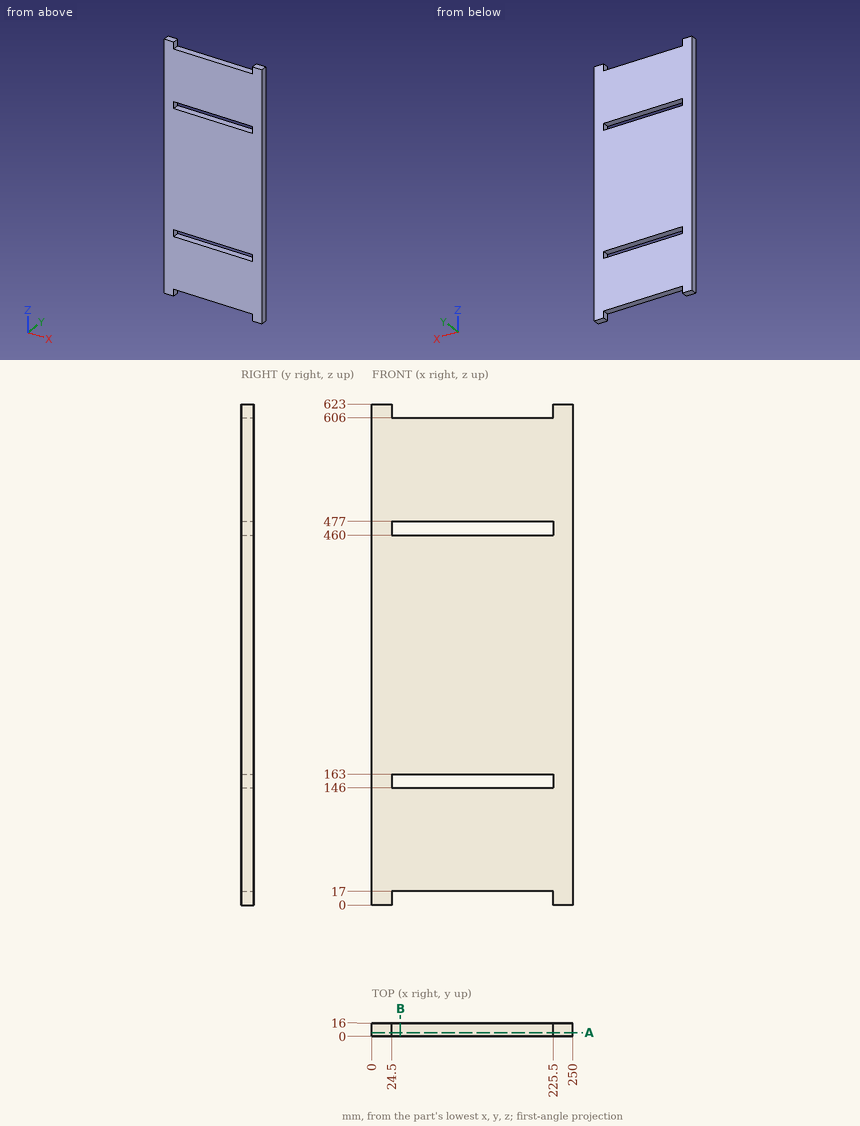
Here's the drawing with two shaded views (mm, measured from the low corner). I have some questions. Give positions to 0.01 mm unless a question says otherwise; leave off trailing zeros. Write each loop counter-clockwise with the first axis right and the second up, starting at its lowest first coordinate (ties: lowest second). Pieces come first, ordered by that corner, then holes. Notation, with made-up numbers: (3, -25.5) -> (29, -25.5) arc R10 cw to (29, -17.5) -> close; hole circle Ø6 at (-35, 5.25). An arc over 180 degrees is marked (long way). Answer as a JSON object with one key per item and string values. Group by question number.
Item 1: I'm going to push flat-ended pins straight in: P1, Ø5, axis at x = 114.5, y = 9.5, coming from the -Z side; P2, Ø1, axis at y = 6, z = 530.5, coming from the -X side; P3, Ø1, axis at x = 191, y = 12, coming from the +Z side. Where does each tip first touch, or does it pass through?
Item 2: Suppose I cut it at A-A (y = 4.25). Please give me the cut outline in (x, z), plus the area to 3 significant figures.
Item 3: Suppose I cut it at B-B (x = 35.5). Please give me the cut outline in (y, z).
Item 4: Please list where this line runs through material, in increasing order: line 1 (Z direction, x = 125.5, y = 14.25). Write a range as [from, to].
Findings:
{
 "1": {"P1": "stops at z = 17", "P2": "stops at x = 0", "P3": "stops at z = 606"},
 "2": {"outline": "(0, 0) -> (24.5, 0) -> (24.5, 17) -> (225.5, 17) -> (225.5, 0) -> (250, 0) -> (250, 623) -> (225.5, 623) -> (225.5, 606) -> (24.5, 606) -> (24.5, 623) -> (0, 623) -> close; hole (24.5, 146) -> (225.5, 146) -> (225.5, 163) -> (24.5, 163) -> close; hole (24.5, 460) -> (225.5, 460) -> (225.5, 477) -> (24.5, 477) -> close", "area": "142,000 mm²"},
 "3": {"outline": "(0, 17) -> (16, 17) -> (16, 146) -> (0, 146) -> close; (0, 163) -> (16, 163) -> (16, 460) -> (0, 460) -> close; (0, 477) -> (16, 477) -> (16, 606) -> (0, 606) -> close"},
 "4": {"line 1": "z = [17, 146], [163, 460], [477, 606]"}
}
